Could you check a few things on this model? Use its own coordinates, in mm. Face numbers are marked on the shaded views. A direction names the side the tool comes from. Coordinates: 2 decimals unless noted, no trailing zeros. Write each loop counter-clockwise with the first axis right and the second up, starting at its lowest first coordinate (ties: lowest second). Pieces come first, ordered by that corner, then holes. Notation, with made-up numbers: M 66.25,28.5 L 107.25,28.5 A22 ccw 107.25,43.5 Z; hole C -23.75,68 d2. An arc over 180 degrees is marked long. Write item = value, one per line.
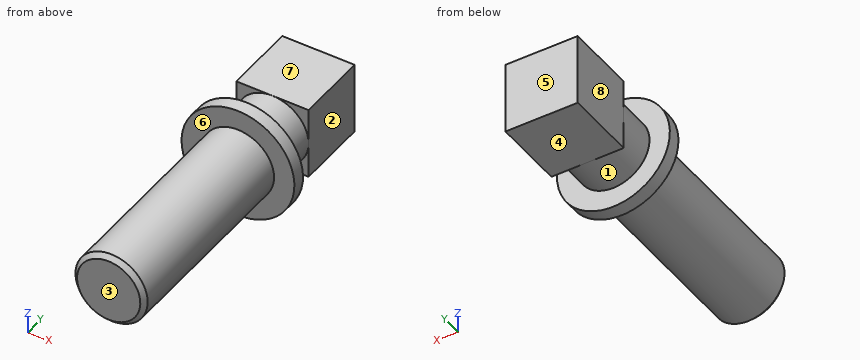
```python
from build123d import *

# Parameters (mm, degrees)
SHANK_SKETCH_16_R          = 8
SHANK_16X45_DEPTH          = 45
SHANK_CHAMFER_1X45_SIZE    = 1
COLLAR_SKETCH_25_R         = 12.5
COLLAR_25X3_DEPTH          = 3
NECK_SKETCH_16_R           = 8
NECK_16X9_DEPTH            = 9
SQUARE_HEAD_SKETCH_16X16_W = 16
SQUARE_HEAD_SKETCH_16X16_H = 16
SQUARE_HEAD_16X16X16_DEPTH = 16


with BuildPart() as part:
    # Shank Sketch Ø16 → Shank Ø16x45 (new body)
    with BuildSketch(Plane(origin=(0, 0, 0), x_dir=(1, 0, 0), z_dir=(0, 1, 0))):
        with Locations(Location((0, 0, 0), (0, 0, 90))):
            Circle(SHANK_SKETCH_16_R)
    extrude(amount=SHANK_16X45_DEPTH)

    # Shank Chamfer 1x45°
    shank_chamfer_1x45_edges = [part.edges().sort_by_distance(p)[0] for p in [
        (0, 0, 8),
    ]]
    chamfer(shank_chamfer_1x45_edges, length=SHANK_CHAMFER_1X45_SIZE)

    # Collar Sketch Ø25 → Collar Ø25x3 (add)
    with BuildSketch(Plane(origin=(0, 45, 0), x_dir=(1, 0, 0), z_dir=(0, 1, 0))):
        with Locations(Location((0, 0, 0), (0, 0, 270))):
            Circle(COLLAR_SKETCH_25_R)
    extrude(amount=COLLAR_25X3_DEPTH)

    # Neck Sketch Ø16 → Neck Ø16x9 (add)
    with BuildSketch(Plane(origin=(0, 48, 0), x_dir=(1, 0, 0), z_dir=(0, 1, 0))):
        with Locations(Location((0, 0, 0), (0, 0, 90))):
            Circle(NECK_SKETCH_16_R)
    extrude(amount=NECK_16X9_DEPTH)

    # Square Head Sketch 16x16 → Square Head 16x16x16 (add)
    with BuildSketch(Plane(origin=(0, 57, 0), x_dir=(1, 0, 0), z_dir=(0, 1, 0))):
        Rectangle(SQUARE_HEAD_SKETCH_16X16_W, SQUARE_HEAD_SKETCH_16X16_H)
    extrude(amount=SQUARE_HEAD_16X16X16_DEPTH)


solid = part.part
```
Item 1: If we mould it in two halves opening along Y, with no side actions, what happens to the marked faces 1, 2 and 3? For each: pulls with the +Y half, pulls with the -Y half, needs draft (parallel to the pull), parting line crosses it, or undercut.
Numbers:
face_1 = undercut
face_2 = needs draft
face_3 = pulls with the -Y half
Item 2: Imagine slicing it at B-B (y = 51). Write out the boundary of the cut face in (x, z), and give its area (3 significant figures).
Numbers:
outline = C 0,0 d16
area = 201 mm²
Item 3: If I drill on line 1 along Y through (x, z) = (7, 5.75); line 2 along Y through (x, z) = (-10.5, -0.5); line 3 along X through (y, z) = (68, 1), over which ranges is the centre line in solid material (lowest first)?
Numbers:
line_1 = 45 to 48, 57 to 73
line_2 = 45 to 48
line_3 = -8 to 8
Item 4: For the marked faces 4, 5, 6, 7 and 8, which set-ups out of +Z, -Z, +X, -X, +Y, -Y let a thin tool reach every point of the face, with its end or its side?
Numbers:
face_4 = -Z, +X, -X, +Y
face_5 = +Z, -Z, +X, -X, +Y
face_6 = -Y
face_7 = +Z, +X, -X, +Y
face_8 = +Z, -Z, -X, +Y
Item 5: Imagine slicing it at A-A (x = -10). Write out the boundary of the cut face in (y, z).
Numbers:
outline = M 45,-7.5 L 48,-7.5 L 48,7.5 L 45,7.5 Z
Item 6: I'm going to push flat-ended pins straight in: P1, Ø8, axis at x = -6.5, y = 28.5, coming from the +Z side; P2, Ø1.5, axis at y = 12.5, z = -7.5, coming from the -X side; P3, Ø13, axis at y = 62, z = -2, coming from the +X side. Where does each tip first touch, or does it pass through?
Numbers:
P1 = 7.6
P2 = -4.29
P3 = 8
